Check sheet for the modelled part. Datum: model origin and axes. Units: mm. A direction names the side the tool comes from. Give positions to 0.01 mm unless a question says otherwise; leave off trailing zeros. Loops run counter-clockwise (first coordinate to the right, second up) from the corner with the lowest first, then second, coordinate; pieces in that order, holes last. Notation, with made-up numbers: (15.25, -19) - (32.25, -19) arc R20 ccw to (32.25, -13) - close; hole circle Ø4 at (39, -26.5). An arc over 180 degrees is marked (long way). Answer in a Markdown table with one row per item. Add a question column.
(1) Sectioned sample at C-C on y = 8. Enter the section's corners in (x, z).
(2) Thickness scan on L1, parallel to X at y = 7.25, z = 51; L2, parallel to Y at x = 51, z = -15; L3, parallel to X at y = 41, z = 0. Record the ranges inside material, lowest first.
(3) Go/stop test with flat-tipped pins: P1, Ø5, axis at y = 32.5, z = 12, coming from the -X side; P2, Ø10, axis at x = 59, z = 54.5, coming from the +Y side; P3, Ø8, axis at x = 12.5, y = 34.5, coming from the +Z side. Record where each tip stops, or that it passes through.
(4) Set-up check for faces 1 (the face through (-31, 40, 0)), 2 (the face through (-45, 40, 19)), 3 (the face through (-63, 34, 14)), 4 (the face through (0, 40, -64)): record each of +Z, -Z, +X, -X, +Y, -Y from which the full face is reachable in a straight line by a thin tool's end or side.
(5) Draft check along Y on faces 5 (the face through (47, 40, 9)), 6 (the face through (59.39, 52.58, -14.07)), 7 (the face through (-55, 47, 14)). Enter one of: released by +Y, released by -Y, zero draft, split by the parting line, or undercut.
(6) Sectioned sample at A-A on x = 0. Enter the section's corners in (y, z), then the cut area to 3 significant figures.
(7) Sectioned sample at D-D on z = -53. Enter the section's corners in (x, y), then the cut area to 3 significant figures.
(8) Sectioned sample at B-B on z = 0. Enter the section's corners in (x, y).
from build123d import *

# Parameters (mm, degrees)
BASE_PLATE_DEPTH              = 25
PLATE_MOUNTING_HOLES_SKETCH_R = 10
PLATE_MOUNTING_HOLES_DEPTH    = 112
CENTRAL_BOSS_DEPTH            = 31
LUG_START                     = -31
LUG_PAIR_A_DEPTH              = 31
LUG_PAIR_B_DEPTH              = 31
LUG_PIN_HOLES_SKETCH_R        = 5
LUG_PIN_HOLES_DEPTH           = 118
LUG_A_FILLET_1_R              = 12
LUG_A_FILLET_2_R              = 12
LUG_B_FILLET_1_R              = 12
LUG_B_FILLET_2_R              = 12
CENTRAL_BORE_SKETCH_R         = 14
CENTRAL_BORE_DEPTH            = 118
BORE_COUNTERBORE_SKETCH_R     = 20
BORE_COUNTERBORE_DEPTH        = 42
BOTTOM_SPIGOT_SKETCH_R        = 56
BOTTOM_SPIGOT_DEPTH           = 6
SPIGOT_BORE_SKETCH_R          = 14
SPIGOT_BORE_DEPTH             = 120
FLANGE_HOLE_1_SKETCH_R        = 10
FLANGE_HOLE_1_DEPTH           = 22
FLANGE_HOLE_2_SKETCH_R        = 10
FLANGE_HOLE_2_DEPTH           = 22


with BuildPart() as part:
    # Base Plate Sketch → Base Plate (new body)
    with BuildSketch(Plane(origin=(0, 0, 0), x_dir=(1, 0, 0), z_dir=(0, 1, 0))):
        with BuildLine():
            Line((77, 0), (77, 51))
            ThreePointArc((77, 51), (69.384776311, 69.384776311), (51, 77))
            Line((51, 77), (-51, 77))
            ThreePointArc((-51, 77), (-69.384776311, 69.384776311), (-77, 51))
            Line((-77, 51), (-77, -51))
            ThreePointArc((-77, -51), (-69.384776311, -69.384776311), (-51, -77))
            Line((-51, -77), (51, -77))
            ThreePointArc((51, -77), (69.384776311, -69.384776311), (77, -51))
            Line((77, -51), (77, 0))
        make_face()
    extrude(amount=BASE_PLATE_DEPTH)

    # Plate Mounting Holes Sketch → Plate Mounting Holes (cut)
    with BuildSketch(Plane(origin=(0, 25, 0), x_dir=(1, 0, 0), z_dir=(0, 1, 0))):
        with Locations(Location((-51, 51, 0), (0, 0, 270))):
            Circle(PLATE_MOUNTING_HOLES_SKETCH_R)
        with Locations(Location((51, 51, 0), (0, 0, 270))):
            Circle(PLATE_MOUNTING_HOLES_SKETCH_R)
        with Locations(Location((51, -51, 0), (0, 0, 270))):
            Circle(PLATE_MOUNTING_HOLES_SKETCH_R)
        with Locations(Location((-51, -51, 0), (0, 0, 270))):
            Circle(PLATE_MOUNTING_HOLES_SKETCH_R)
    extrude(amount=-PLATE_MOUNTING_HOLES_DEPTH, mode=Mode.SUBTRACT)

    # Central Boss Sketch → Central Boss (add)
    with BuildSketch(Plane(origin=(0, 25, 0), x_dir=(1, 0, 0), z_dir=(0, 1, 0))):
        with BuildLine():
            Line((14.551173168, 56.595440502), (29.545654505, 9.383725265))
            ThreePointArc((29.545654505, 9.383725265), (30.89470992, 2.552821763), (30.685167625, -4.406868258))
            Line((30.685167625, -4.406868258), (14.551173168, -56.595440502))
            ThreePointArc((14.551173168, -56.595440502), (-3.070625216, -63.736156878), (-17.266235066, -51.086956522))
            Line((-17.266235066, -51.086956522), (-29.736293724, -8.760869565))
            ThreePointArc((-29.736293724, -8.760869565), (-30.998289096, 0.325688707), (-29.545654505, 9.383725265))
            Line((-29.545654505, 9.383725265), (-14.551173168, 56.595440502))
            ThreePointArc((-14.551173168, 56.595440502), (0, 64), (14.551173168, 56.595440502))
        make_face()
    extrude(amount=CENTRAL_BOSS_DEPTH)

    # Lug Pair A Sketch → Lug Pair A (add)
    with BuildSketch(Plane(origin=(0, 56, 0), x_dir=(1, 0, 0), z_dir=(0, 1, 0)).offset(LUG_START)):
        with BuildLine():
            Line((31, 0), (31, 9))
            Line((31, 9), (63, 9))
            Line((63, 9), (63, 19))
            Line((63, 19), (31, 19))
            Line((31, 19), (26.491517384, 19))
            Line((26.491517384, 19), (29.545654505, 9.383725265))
            ThreePointArc((29.545654505, 9.383725265), (30.634256068, 4.747879018), (31, 0))
        make_face()
        with BuildLine():
            Line((31, -9), (31, 0))
            ThreePointArc((31, 0), (30.921191733, -2.209049981), (30.685167625, -4.406868258))
            ThreePointArc((30.685167625, -4.406868258), (29.6170045, -9.156038686), (27.818568264, -13.679446617))
            Line((27.818568264, -13.679446617), (26.173729651, -19))
            Line((26.173729651, -19), (31, -19))
            Line((31, -19), (63, -19))
            Line((63, -19), (63, -9))
            Line((63, -9), (31, -9))
        make_face()
        with BuildLine():
            ThreePointArc((24.494897428, 19), (27.444735347, 14.414801481), (29.545654505, 9.383725265))
            Line((29.545654505, 9.383725265), (26.491517384, 19))
            Line((26.491517384, 19), (24.494897428, 19))
        make_face()
        with BuildLine():
            Line((26.173729651, -19), (27.818568264, -13.679446617))
            ThreePointArc((27.818568264, -13.679446617), (26.29166684, -16.424014575), (24.494897428, -19))
            Line((24.494897428, -19), (26.173729651, -19))
        make_face()
        with BuildLine():
            ThreePointArc((27.818568264, -13.679446617), (29.6170045, -9.156038686), (30.685167625, -4.406868258))
            Line((30.685167625, -4.406868258), (27.818568264, -13.679446617))
        make_face()
    extrude(amount=LUG_PAIR_A_DEPTH)

    # Lug Pair B Sketch → Lug Pair B (add)
    with BuildSketch(Plane(origin=(0, 56, 0), x_dir=(1, 0, 0), z_dir=(0, 1, 0)).offset(LUG_START)):
        with BuildLine():
            ThreePointArc((-29.736293724, -8.760869565), (-30.682446981, -4.425770811), (-31, 0))
            Line((-31, 0), (-31, -9))
            Line((-31, -9), (-63, -9))
            Line((-63, -9), (-63, -19))
            Line((-63, -19), (-26.719653956, -19))
            Line((-26.719653956, -19), (-29.736293724, -8.760869565))
        make_face()
        with BuildLine():
            Line((-31, 9), (-31, 0))
            ThreePointArc((-31, 0), (-30.634256068, 4.747879018), (-29.545654505, 9.383725265))
            Line((-29.545654505, 9.383725265), (-26.491517384, 19))
            Line((-26.491517384, 19), (-63, 19))
            Line((-63, 19), (-63, 9))
            Line((-63, 9), (-31, 9))
        make_face()
        with BuildLine():
            ThreePointArc((-24.494897428, -19), (-27.594663822, -14.125669136), (-29.736293724, -8.760869565))
            Line((-29.736293724, -8.760869565), (-26.719653956, -19))
            Line((-26.719653956, -19), (-24.494897428, -19))
        make_face()
        with BuildLine():
            Line((-26.491517384, 19), (-29.545654505, 9.383725265))
            ThreePointArc((-29.545654505, 9.383725265), (-27.444735347, 14.414801481), (-24.494897428, 19))
            Line((-24.494897428, 19), (-26.491517384, 19))
        make_face()
    extrude(amount=LUG_PAIR_B_DEPTH)

    # Lug Pin Holes Sketch → Lug Pin Holes (cut)
    with BuildSketch(Plane.XY.offset(19)):
        with Locations((51, 44)):
            Circle(LUG_PIN_HOLES_SKETCH_R)
        with Locations((-51, 44)):
            Circle(LUG_PIN_HOLES_SKETCH_R)
    extrude(amount=-LUG_PIN_HOLES_DEPTH, mode=Mode.SUBTRACT)

    # Lug A Fillet 1
    lug_a_fillet_1_edges = [part.edges().sort_by_distance(p)[0] for p in [
        (63, 56, 14),
    ]]
    fillet(lug_a_fillet_1_edges, radius=LUG_A_FILLET_1_R)

    # Lug A Fillet 2
    lug_a_fillet_2_edges = [part.edges().sort_by_distance(p)[0] for p in [
        (63, 56, -14),
    ]]
    fillet(lug_a_fillet_2_edges, radius=LUG_A_FILLET_2_R)

    # Lug B Fillet 1
    lug_b_fillet_1_edges = [part.edges().sort_by_distance(p)[0] for p in [
        (-63, 56, -14),
    ]]
    fillet(lug_b_fillet_1_edges, radius=LUG_B_FILLET_1_R)

    # Lug B Fillet 2
    lug_b_fillet_2_edges = [part.edges().sort_by_distance(p)[0] for p in [
        (-63, 56, 14),
    ]]
    fillet(lug_b_fillet_2_edges, radius=LUG_B_FILLET_2_R)

    # Central Bore Sketch → Central Bore (cut)
    with BuildSketch(Plane(origin=(0, 56, 0), x_dir=(1, 0, 0), z_dir=(0, 1, 0))):
        with Locations(Location((0, 0, 0), (0, 0, 270))):
            Circle(CENTRAL_BORE_SKETCH_R)
    extrude(amount=-CENTRAL_BORE_DEPTH, mode=Mode.SUBTRACT)

    # Bore Counterbore Sketch → Bore Counterbore (cut)
    with BuildSketch(Plane(origin=(0, 56, 0), x_dir=(1, 0, 0), z_dir=(0, 1, 0))):
        with Locations(Location((0, 0, 0), (0, 0, 270))):
            Circle(BORE_COUNTERBORE_SKETCH_R)
    extrude(amount=-BORE_COUNTERBORE_DEPTH, mode=Mode.SUBTRACT)

    # Bottom Spigot Sketch → Bottom Spigot (add)
    with BuildSketch(Plane.XZ):
        with Locations(Location((0, 0, 0), (0, 0, 270))):
            Circle(BOTTOM_SPIGOT_SKETCH_R)
    extrude(amount=BOTTOM_SPIGOT_DEPTH)

    # Spigot Bore Sketch → Spigot Bore (cut)
    with BuildSketch(Plane(origin=(0, 0, 0), x_dir=(1, 0, 0), z_dir=(0, 1, 0))):
        with Locations(Location((0, 0, 0), (0, 0, 270))):
            Circle(SPIGOT_BORE_SKETCH_R)
    extrude(amount=-SPIGOT_BORE_DEPTH, mode=Mode.SUBTRACT)

    # Flange Hole 1 Sketch → Flange Hole 1 (cut)
    with BuildSketch(Plane(origin=(0, 56, 0), x_dir=(1, 0, 0), z_dir=(0, 1, 0))):
        with Locations(Location((0, 46, 0), (0, 0, 270))):
            Circle(FLANGE_HOLE_1_SKETCH_R)
    extrude(amount=-FLANGE_HOLE_1_DEPTH, mode=Mode.SUBTRACT)

    # Flange Hole 2 Sketch → Flange Hole 2 (cut)
    with BuildSketch(Plane(origin=(0, 56, 0), x_dir=(1, 0, 0), z_dir=(0, 1, 0))):
        with Locations(Location((0, -46, 0), (0, 0, 270))):
            Circle(FLANGE_HOLE_2_SKETCH_R)
    extrude(amount=-FLANGE_HOLE_2_DEPTH, mode=Mode.SUBTRACT)


solid = part.part
Reply:
| question | item | result |
|---|---|---|
| 1 | outline | (-77, -51) arc R26 ccw to (-51, -77) - (51, -77) arc R26 ccw to (77, -51) - (77, 51) arc R26 ccw to (51, 77) - (-51, 77) arc R26 ccw to (-77, 51) - close; hole circle Ø20 at (-51, -51); hole circle Ø20 at (-51, 51); hole circle Ø28 at (0, 0); hole circle Ø20 at (51, -51); hole circle Ø20 at (51, 51) |
| 2 | L1 | -77 to -61, -41 to 41, 61 to 77 |
| 2 | L2 | -6 to 39, 49 to 56 |
| 2 | L3 | -31 to -20, 20 to 31 |
| 3 | P1 | x = -63 |
| 3 | P2 | y = 25 |
| 3 | P3 | z = 61.87 |
| 4 | face 1 | -X, +Y |
| 4 | face 2 | +Z, -X, +Y |
| 4 | face 3 | +Z, -Z, -X, +Y |
| 4 | face 4 | -Z, +Y |
| 5 | face 5 | zero draft |
| 5 | face 6 | released by +Y |
| 5 | face 7 | undercut |
| 6 | outline | (-6, -56) - (0, -56) - (0, -77) - (25, -77) - (25, -64) - (56, -64) - (56, -56) - (34, -56) - (34, -36) - (56, -36) - (56, -20) - (14, -20) - (14, -14) - (-6, -14) - close; (-6, 14) - (14, 14) - (14, 20) - (56, 20) - (56, 36) - (34, 36) - (34, 56) - (56, 56) - (56, 64) - (25, 64) - (25, 77) - (0, 77) - (0, 56) - (-6, 56) - close |
| 6 | area | 5,370 mm^2 |
| 7 | outline | (-76.92, 0) - (-60.8, 0) - (-60.8, 25) - (-76.92, 25) - close; (-41.2, 0) - (-18.08, 0) - (-18.08, -6) - (18.08, -6) - (18.08, 0) - (41.2, 0) - (41.2, 25) - (15.69, 25) - (15.69, 56) - (7.14, 56) - (7.14, 34) - (-7.14, 34) - (-7.14, 56) - (-15.69, 56) - (-15.69, 25) - (-41.2, 25) - close; (60.8, 0) - (76.92, 0) - (76.92, 25) - (60.8, 25) - close |
| 7 | area | 3,740 mm^2 |
| 8 | outline | (-77, 0) - (-56, 0) - (-56, -6) - (-14, -6) - (-14, 14) - (-20, 14) - (-20, 56) - (-31, 56) - (-31, 25) - (-77, 25) - close; (14, -6) - (56, -6) - (56, 0) - (77, 0) - (77, 25) - (31, 25) - (31, 56) - (20, 56) - (20, 14) - (14, 14) - close |
